Can you work these out from the model? Positions are in its coordinate system, mm. Round coordinates to 2 decimals unless told otherwise and drop trailing zeros. Loops run counter-clockwise (first coordinate to the right, second up) from the corner with the lowest first, then second, coordinate; pieces in that order, holes last. Notation, with made-up numbers: (84.5, -4.5) -> (120.5, -4.5) arc R33 cw to (120.5, 28.5) -> close; hole circle Ø1 at (47, -37). An arc over 180 degrees is marked (long way). Use a Markdown table: item, result.
from build123d import *

# Parameters (mm, degrees)
SKETCH_1_W          = 440
SKETCH_1_H          = 292
EXTRUDE_1_DEPTH     = 60
CUT_EXTRUDE_1_DEPTH = 379
CUT_EXTRUDE_2_DEPTH = 467
SKETCH_5_R          = 2.5
CUT_EXTRUDE_3_DEPTH = 20


with BuildPart() as part:
    # 草图1 → 凸台-拉伸1 (new body)
    with BuildSketch(Plane(origin=(0, 0, 0), x_dir=(1, 0, 0), z_dir=(0, 1, 0))):
        with Locations((220, 146)):
            Rectangle(SKETCH_1_W, SKETCH_1_H)
    extrude(amount=EXTRUDE_1_DEPTH)

    # 草图3 → 切除-拉伸1 (cut)
    with BuildSketch(Plane(origin=(0, 0, -292), x_dir=(-1, 0, 0), z_dir=(0, 0, -1))):
        Polygon((-440, 60), (-440, 25), (-360, 60), align=None)
        Polygon((-80, 60), (0, 25), (0, 60), align=None)
    extrude(amount=-CUT_EXTRUDE_1_DEPTH, mode=Mode.SUBTRACT)

    # 草图4 → 切除-拉伸2 (cut)
    with BuildSketch(Plane.ZY):
        Polygon((-292, 60), (-292, 25), (-222, 60), align=None)
        Polygon((-70, 60), (0, 25), (0, 60), align=None)
    extrude(amount=-CUT_EXTRUDE_2_DEPTH, mode=Mode.SUBTRACT)

    # 草图5 → 切除-拉伸3 (cut)
    with BuildSketch(Plane(origin=(0, 60, 0), x_dir=(1, 0, 0), z_dir=(0, 1, 0))):
        with Locations(Location((270, 196, 0), (0, 0, 270))):
            Circle(SKETCH_5_R)
        with Locations(Location((257.5, 183.5, 0), (0, 0, 270))):
            Circle(SKETCH_5_R)
        with Locations(Location((270, 96, 0), (0, 0, 270))):
            Circle(SKETCH_5_R)
        with Locations(Location((257.5, 108.5, 0), (0, 0, 270))):
            Circle(SKETCH_5_R)
        with Locations(Location((170, 96, 0), (0, 0, 270))):
            Circle(SKETCH_5_R)
        with Locations(Location((182.5, 108.5, 0), (0, 0, 270))):
            Circle(SKETCH_5_R)
        with Locations(Location((170, 196, 0), (0, 0, 270))):
            Circle(SKETCH_5_R)
        with Locations(Location((182.5, 183.5, 0), (0, 0, 270))):
            Circle(SKETCH_5_R)
    extrude(amount=-CUT_EXTRUDE_3_DEPTH, mode=Mode.SUBTRACT)


solid = part.part
1. I want a section at A-A (z = -79.5). Please give me the cut outline in (x, y).
Answer sheet:
| item | result |
|---|---|
| outline | (0, 0) -> (440, 0) -> (440, 25) -> (360, 60) -> (80, 60) -> (0, 25) -> close |
2. Will these pins go through, and if not, where does the flat tip stop? pin 1 Ø4 at (y, z) = (32.5, -76.5) entering from +X; pin 2 Ø5 at (x, y) = (238, 50.5) entering from -Z; pin 3 Ø2.5 at (x, z) = (169, -96.5) entering from +Y.
Answer sheet:
| item | result |
|---|---|
| pin 1 | stops at x = 427.43 |
| pin 2 | stops at z = -246 |
| pin 3 | stops at y = 40 |
3. I want a section at B-B (x = 92.5). Please give me the cut outline in (y, z).
Answer sheet:
| item | result |
|---|---|
| outline | (0, -292) -> (25, -292) -> (60, -222) -> (60, -70) -> (25, 0) -> (0, 0) -> close |
4. I need wall thicknesses on line 1 (Z direction, x = 182.5, y = 51); line 2 (X direction, y = 50, z = -196); line 3 (X direction, y = 54.75, z = -183.5). Which ranges of each line are inside material? Lowest first, please.
Answer sheet:
| item | result |
|---|---|
| line 1 | z = -240 to -186, -181 to -111, -106 to -52 |
| line 2 | x = 57.14 to 167.5, 172.5 to 267.5, 272.5 to 382.86 |
| line 3 | x = 68 to 180, 185 to 255, 260 to 372 |
